Could you check a few things on this drawing? It's one solid part, dimensions in mm from its lowest x, y, z. A direction names the side the tool comes from. Give positions to 0.01 mm unless a question says otherwise; leave off trailing zeros. Order: outer loops, then holes, each group sorted by start corner. A loop starts at its lowest first (then second) coordinate and runs counter-clockwise, first axis right, second up.
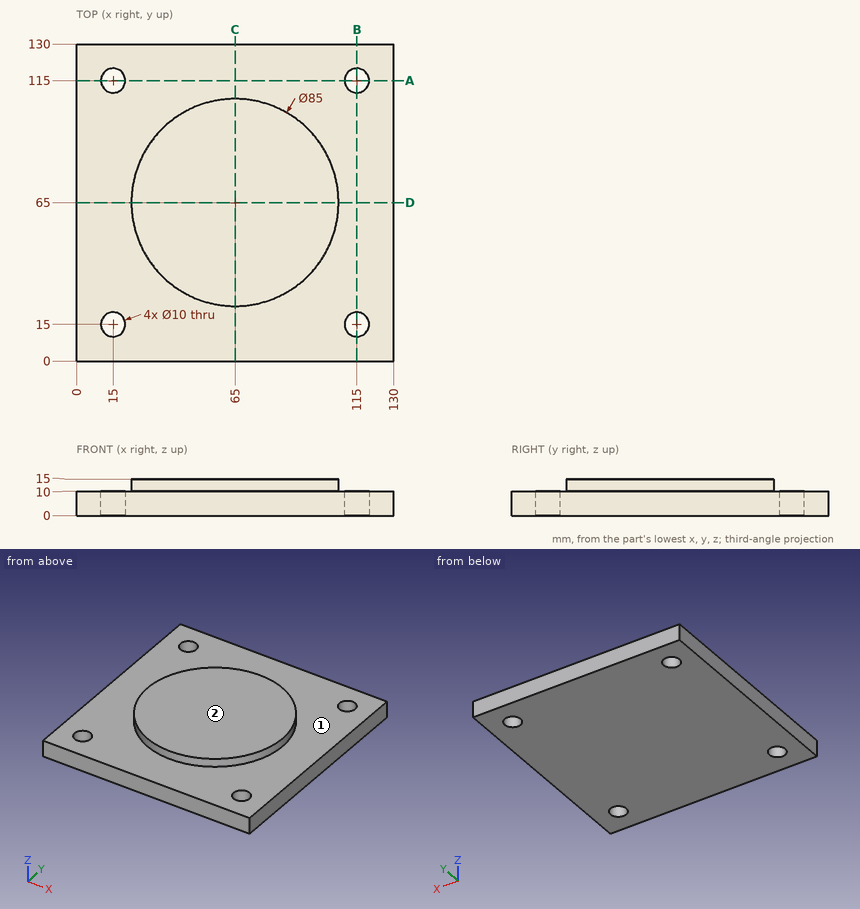
Item 1: Imagine slicing it at A-A on y = 115. List the corners of the cut face in (x, z) for me.
Findings:
outline: (0, 0) - (10, 0) - (10, 10) - (0, 10) - close; (20, 0) - (110, 0) - (110, 10) - (20, 10) - close; (120, 0) - (130, 0) - (130, 10) - (120, 10) - close
Item 2: Please list where these lines run through material, in increasing order: line 1 along Y through (x, z) = (15, 6.5); line 2 along Y through (x, z) = (16, 5.5); line 3 along Z through (x, y) = (44.5, 113).
Findings:
line 1: y = 0 to 10, 20 to 110, 120 to 130
line 2: y = 0 to 10.1, 19.9 to 110.1, 119.9 to 130
line 3: z = 0 to 10
Item 3: For pin 1 (10 mm diameter, centred on x = 81.5, y = 19, fed in from +Z), with a flat end and sliding along its axis, tell me the tip position at first contact or that it passes through.
Findings:
pin 1: stops at z = 10
Item 4: For the marked faces 1 and 2, which set-ups out of +Z, -Z, +X, -X, +Y, -Y let a thin tool reach every point of the face, with its end or its side?
Findings:
face 1: +Z
face 2: +Z, +X, -X, +Y, -Y
Item 5: Imagine slicing it at C-C on x = 65. List the corners of the cut face in (y, z) for me.
Findings:
outline: (0, 0) - (130, 0) - (130, 10) - (107.5, 10) - (107.5, 15) - (22.5, 15) - (22.5, 10) - (0, 10) - close
